Design review of the part built by this model. Coordinates are the model's own, in mm. A direction names the side the tool comes from. Coordinates: 2 decimals unless noted, no trailing zeros. Order: outer loops, then holes, each group sorted by start corner. A loop starts at its lowest first (then second) coordinate and runs counter-clockwise, first axis right, second up. Notation, with made-up numbers: M 6,-40 L 44,-40 A17 ccw 44,-26 Z; hole C -18.5,13 d11. An arc over 180 degrees is marked long. Answer as a JSON object with one key per item and string values.
from build123d import *

# Parameters (mm, degrees)
MOUNTING_FLANGE_DEPTH    = 10
HOUSING_BLOCK_PROFILE_W  = 30
HOUSING_BLOCK_PROFILE_H  = 30
HOUSING_BLOCK_DEPTH      = 30
UPPER_BLOCK_PROFILE_W    = 8
UPPER_BLOCK_PROFILE_H    = 30
UPPER_BLOCK_DEPTH        = 26
SIDE_RELIEF_CUT_DEPTH    = 8
GUSSET_A_DEPTH           = 10
GUSSET_B_DEPTH           = 10
MOUNTING_HOLES_PROFILE_R = 1
MOUNTING_HOLES_4X_DEPTH  = 10
COUNTERBORE_25_PROFILE_R = 12.5
COUNTERBORE_25_DEPTH     = 8
BORE_13_PROFILE_R        = 6.5
BORE_13_DEPTH            = 8


with BuildPart() as part:
    # Flange Profile → Mounting Flange (new body)
    with BuildSketch(Plane.XY):
        with BuildLine():
            Line((3, 0), (71, 0))
            ThreePointArc((71, 0), (73.121320344, 0.878679656), (74, 3))
            Line((74, 3), (74, 37))
            ThreePointArc((74, 37), (73.121320344, 39.121320344), (71, 40))
            Line((71, 40), (3, 40))
            ThreePointArc((3, 40), (0.878679656, 39.121320344), (0, 37))
            Line((0, 37), (0, 25))
            Line((0, 25), (12, 25))
            ThreePointArc((12, 25), (17, 20), (12, 15))
            Line((12, 15), (0, 15))
            Line((0, 15), (0, 3))
            ThreePointArc((0, 3), (0.878679656, 0.878679656), (3, 0))
        make_face()
    extrude(amount=MOUNTING_FLANGE_DEPTH)

    # Housing Block Profile → Housing Block (add)
    with BuildSketch(Plane.XY.offset(10)):
        with Locations((53, 20)):
            Rectangle(HOUSING_BLOCK_PROFILE_W, HOUSING_BLOCK_PROFILE_H)
    extrude(amount=HOUSING_BLOCK_DEPTH)

    # Upper Block Profile → Upper Block (add)
    with BuildSketch(Plane.ZY.offset(-38)):
        with Locations((14, 20)):
            Rectangle(UPPER_BLOCK_PROFILE_W, UPPER_BLOCK_PROFILE_H)
    extrude(amount=UPPER_BLOCK_DEPTH)

    # Side Relief Profile → Side Relief Cut (cut)
    with BuildSketch(Plane(origin=(0, 0, 10), x_dir=(-1, 0, 0), z_dir=(0, 0, -1))):
        with BuildLine():
            Line((-12, 25), (-12, 15))
            ThreePointArc((-12, 15), (-17, 20), (-12, 25))
        make_face()
    extrude(amount=-SIDE_RELIEF_CUT_DEPTH, mode=Mode.SUBTRACT)

    # Gusset A Profile → Gusset A (add)
    with BuildSketch(Plane.XZ.offset(-5)):
        Polygon((12, 10), (12, 18), (0, 10), align=None)
    extrude(amount=-GUSSET_A_DEPTH)

    # Gusset B Profile → Gusset B (add)
    with BuildSketch(Plane(origin=(0, 35, 0), x_dir=(1, 0, 0), z_dir=(0, 1, 0))):
        Polygon((12, -18), (12, -10), (0, -10), align=None)
    extrude(amount=-GUSSET_B_DEPTH)

    # Mounting Holes Profile → Mounting Holes 4x (cut)
    with BuildSketch(Plane.XY.offset(10)):
        with Locations((3, 37)):
            Circle(MOUNTING_HOLES_PROFILE_R)
        with Locations((71, 37)):
            Circle(MOUNTING_HOLES_PROFILE_R)
        with Locations((71, 3)):
            Circle(MOUNTING_HOLES_PROFILE_R)
        with Locations((3, 3)):
            Circle(MOUNTING_HOLES_PROFILE_R)
    extrude(amount=-MOUNTING_HOLES_4X_DEPTH, mode=Mode.SUBTRACT)

    # Counterbore Ø25 Profile → Counterbore Ø25 (cut)
    with BuildSketch(Plane.XY.offset(40)):
        with Locations((53, 20)):
            Circle(COUNTERBORE_25_PROFILE_R)
    extrude(amount=-COUNTERBORE_25_DEPTH, mode=Mode.SUBTRACT)

    # Bore Ø13 Profile → Bore Ø13 (cut)
    with BuildSketch(Plane.XY.offset(32)):
        with Locations((53, 20)):
            Circle(BORE_13_PROFILE_R)
    extrude(amount=-BORE_13_DEPTH, mode=Mode.SUBTRACT)


solid = part.part
1) Tool access review of faces 5 (the flat face through (49, 5, 22)), 6 (the flat face through (68, 20, 25)), 7 (the flat face through (6, 25, 7)), 8 (the flat face through (6, 10, 14)), 9 (the flat face through (53, 20, 24)): name each direction out of +Z, -Z, +X, -X, +Y, -Y from which nothing blocks a thin tool from reaching the whole face with its end or side.
Taken from the geometry:
{"face 5": "+Z, +X, -X, -Y", "face 6": "+Z, +X, +Y, -Y", "face 7": "+Z, -Z, -X", "face 8": "+Z, -X, +Y, -Y", "face 9": "+Z"}
2) Add section B-B (z = 26). State the section outline as (x, y) points, and give its area (3 significant figures).
Taken from the geometry:
{"outline": "M 38,5 L 68,5 L 68,35 L 38,35 Z; hole C 53,20 d13", "area": "767 mm2"}
3) To check wall thickness, follow L1, parallel to Y at x = 71, z = 7.5; L2, parallel to Y at x = 3, z = 6; L3, parallel to Y at x = 53, z = 27. State the ranges of each line that lie inside material, in increasing order.
Taken from the geometry:
{"L1": "y = 0 to 2, 4 to 36, 38 to 40", "L2": "y = 0 to 2, 4 to 15, 25 to 36, 38 to 40", "L3": "y = 5 to 13.5, 26.5 to 35"}
4) Mouldability with a two-part tool opening along Y and no side actions: class faces 1 (the cylindrical face through (73.1, 0.86, 4.93)), 2 (the cylindrical face through (73.14, 39.1, 4.93)), 3 (the cylindrical face through (59.2, 21.95, 28.06)), 4 (the flat face through (0, 31, 5)) as released by +Y, released by -Y, zero draft, split by the parting line, or undercut.
Taken from the geometry:
{"face 1": "released by -Y", "face 2": "released by +Y", "face 3": "undercut", "face 4": "zero draft"}
5) Add section C-C (x = 53). State the section outline as (y, z) points.
Taken from the geometry:
{"outline": "M 0,0 L 40,0 L 40,10 L 35,10 L 35,40 L 32.5,40 L 32.5,32 L 26.5,32 L 26.5,24 L 13.5,24 L 13.5,32 L 7.5,32 L 7.5,40 L 5,40 L 5,10 L 0,10 Z"}
6) Add section D-D (z = 3). State the section outline as (x, y) points, and give its area (3 significant figures).
Taken from the geometry:
{"outline": "M 0,3 A3 ccw 3,0 L 71,0 A3 ccw 74,3 L 74,37 A3 ccw 71,40 L 3,40 A3 ccw 0,37 L 0,25 L 12,25 A5 cw 12,15 L 0,15 Z; hole C 3,3 d2; hole C 3,37 d2; hole C 71,3 d2; hole C 71,37 d2", "area": "2,780 mm2"}
7) Add section A-A (x = 10.5). State the section outline as (y, z) points, and give its area (3 significant figures).
Taken from the geometry:
{"outline": "M 0,0 L 15,0 L 15,17 L 5,17 L 5,10 L 0,10 Z; M 25,0 L 40,0 L 40,10 L 35,10 L 35,17 L 25,17 Z", "area": "440 mm2"}
8) Insertion check: pin 1 Ø10 at (y, z) = (28.5, 20.5) entering from +X; pin 2 Ø6 at (x, z) = (7, 12.5) entering from -Y; pin 3 Ø24 at (y, z) = (22.5, 24.5) entering from -X; pin 4 Ø12 at (x, y) = (30.5, 26) entering from +Z. Each pin has a flat end and moves straight along its axis. Give the tip position at first contact, or say it passes through.
Taken from the geometry:
{"pin 1": "stops at x = 68", "pin 2": "stops at y = 0", "pin 3": "stops at x = 4.14", "pin 4": "stops at z = 18"}
